Geometry: final body of the model. Coordinates: model frame, mm. A direction names the side the tool comes from. Round coordinates to 2 decimals unless told otherwise and drop trailing zeros. Loops run counter-clockwise (first coordinate to the right, second up) from the corner with the lowest first, then second, coordinate; pieces in that order, holes last. Notation, with made-up numbers: (75.25, 84.25) -> (107.25, 84.25) arc R6 cw to (107.25, 88.25) -> close; hole circle Ø9 at (50, 47.5). An arc over 180 degrees is marked (long way). Answer in a Markdown table with one row per item.
```python
from build123d import *


with BuildPart() as part:
    # Sketch1 → Revolve1 (revolve)
    with BuildSketch(Plane.XY, mode=Mode.PRIVATE) as revolve1_sk:
        with BuildLine():
            Line((0, 0), (0, 7.5))
            Line((0, 7.5), (30, 7.5))
            Line((30, 7.5), (30, 5.431390246))
            ThreePointArc((30, 5.431390246), (30.860121025, 4.119849947), (32.405787349, 4.386048651))
            ThreePointArc((32.405787349, 4.386048651), (38.891100593, 5.502966287), (42.5, 0))
            Line((42.5, 0), (0, 0))
        make_face()
    revolve(revolve1_sk.sketch.rotate(Axis((0, 0, 0), (1, 0, 0)), 90), axis=Axis((0, 0, 0), (1, 0, 0)))

    # Sketch2 → Cut-Revolve1 (revolve, cut)
    with BuildSketch(Plane.XY, mode=Mode.PRIVATE) as cut_revolve1_sk:
        Polygon((0, 0), (25, 0), (27.309401077, 0), (37, 0), (47.95408822, 0), (47.95408822, 0.5), (37, 0.5), (37, 1), (27.309401077, 1), (25, 5), (0, 5), align=None)
    revolve(cut_revolve1_sk.sketch.rotate(Axis((0, 0, 0), (1, 0, 0)), 90), axis=Axis((0, 0, 0), (1, 0, 0)), mode=Mode.SUBTRACT)


solid = part.part
```
Item 1: First-contact query: P1, Ø0.6, axis at y = 0, z = 0.5, coming from the -X side; P2, Ø1.5, axis at x = 13.5, y = 4.5, coming from the +Z side; P3, Ø6, axis at y = -5.5, z = 1, coming from the +X side. Flat tips, straight axial feed; report the tip coordinate or a pass-through.
Ans:
| item | result |
|---|---|
| P1 | x = 37 |
| P2 | z = 6.5 |
| P3 | x = 41.91 |
Item 2: Ray query, L1, parallel to Y at x = 16, z = 0; L2, parallel to X at y = 3.75, z = 4.75; L3, parallel to X at y = 0.75, z = -4.5. Return the intervals inside material, ascending.
Ans:
| item | result |
|---|---|
| L1 | -7.5 to -5, 5 to 7.5 |
| L2 | 0 to 30 |
| L3 | 25.25 to 30.29, 32.6 to 40.4 |
Item 3: Section query C-C, the plane x = 15. Output: boundary loops of the cut face in (y, z), and give its area (3 significant figures).
Ans:
| item | result |
|---|---|
| outline | circle Ø15 at (0, 0); hole circle Ø10 at (0, 0) |
| area | 98.2 mm2 |
Item 4: Set-up query: faces 5 (the flat face through (0, 5, -2)), 6 (the cylindrical face through (32, 1, 0)). Return all of +Z, -Z, +X, -X, +Y, -Y with unobstructed straight access to the full face (end or side cutting, diameter ignored); none if empty.
Ans:
| item | result |
|---|---|
| face 5 | +Z, -Z, -X, +Y, -Y |
| face 6 | -X |
Item 5: Mould query, pull axis Y, two halves, no side actions, for faces 1 (the flat face through (30, -4, 4)), 2 (the cylindrical face through (12, 0, -5)), 3 (the cylindrical face through (39.701, 0.488, -0.108)), 4 (the cylindrical face through (15.21, -6.324, 4.032)). Classes: released by +Y, released by -Y, zero draft, split by the parting line, or undercut.
Ans:
| item | result |
|---|---|
| face 1 | zero draft |
| face 2 | undercut |
| face 3 | undercut |
| face 4 | split by the parting line |
Item 6: Section query A-A, the plane y = 0. Output: boundary loops of the cut face in (x, z).
Ans:
| item | result |
|---|---|
| outline | (0, -7.5) -> (30, -7.5) -> (30, -5.43) arc R1.43 cw to (32.41, -4.39) arc R6 ccw to (42.48, -0.5) -> (37, -0.5) -> (37, -1) -> (27.31, -1) -> (25, -5) -> (0, -5) -> close; (0, 5) -> (25, 5) -> (27.31, 1) -> (37, 1) -> (37, 0.5) -> (42.48, 0.5) arc R6 ccw to (32.41, 4.39) arc R1.43 cw to (30, 5.43) -> (30, 7.5) -> (0, 7.5) -> close |
Item 7: Section query D-D, the plane x = 39. Output: boundary loops of the cut face in (y, z), and give its area (3 significant figures).
Ans:
| item | result |
|---|---|
| outline | circle Ø10.91 at (0, 0); hole circle Ø1 at (0, 0) |
| area | 92.7 mm2 |
